from build123d import *

# Parameters (mm, degrees)
BASE_PLATE_DEPTH     = 10
GUIDE_WALL_DEPTH     = 40
HUB_BLOCK_DEPTH      = 40
CLEVIS_START         = -10
CLEVIS_EAR_DEPTH     = 10
GUSSET_SKETCH_W      = 4
GUSSET_SKETCH_H      = 40
GUSSET_DEPTH         = 90
CROSS_HOLE_SKETCH_R  = 8
CROSS_HOLE_16_DEPTH  = 90
HUB_BOSS_SKETCH_R    = 30
HUB_BOSS_60_DEPTH    = 20
HUB_RECESS_SKETCH_R  = 20
HUB_RECESS_40_DEPTH  = 10
SPLINE_BORE_6X_DEPTH = 90


with BuildPart() as part:
    # Base Plate Sketch → Base Plate (new body)
    with BuildSketch(Plane(origin=(0, 0, 0), x_dir=(1, 0, 0), z_dir=(0, 1, 0))):
        with BuildLine():
            Line((-60.5, 45), (60.5, 45))
            ThreePointArc((60.5, 45), (67.571067812, 42.071067812), (70.5, 35))
            Line((70.5, 35), (70.5, -35))
            ThreePointArc((70.5, -35), (67.571067812, -42.071067812), (60.5, -45))
            Line((60.5, -45), (-60.5, -45))
            ThreePointArc((-60.5, -45), (-67.571067812, -42.071067812), (-70.5, -35))
            Line((-70.5, -35), (-70.5, -10))
            Line((-70.5, -10), (-50.5, -10))
            Line((-50.5, -10), (-50.5, 10))
            Line((-50.5, 10), (-70.5, 10))
            Line((-70.5, 10), (-70.5, 35))
            ThreePointArc((-70.5, 35), (-67.571067812, 42.071067812), (-60.5, 45))
        make_face()
    extrude(amount=BASE_PLATE_DEPTH)

    # Guide Wall Sketch → Guide Wall (add)
    with BuildSketch(Plane(origin=(0, 10, 0), x_dir=(1, 0, 0), z_dir=(0, 1, 0))):
        with BuildLine():
            Line((-29.5, 45), (-60.5, 45))
            ThreePointArc((-60.5, 45), (-67.571067812, 42.071067812), (-70.5, 35))
            Line((-70.5, 35), (-70.5, 10))
            Line((-70.5, 10), (-60.5, 10))
            Line((-60.5, 10), (-60.5, 35))
            Line((-60.5, 35), (-29.5, 35))
            Line((-29.5, 35), (-29.5, 45))
        make_face()
        with BuildLine():
            Line((-70.5, -10), (-70.5, -35))
            ThreePointArc((-70.5, -35), (-67.571067812, -42.071067812), (-60.5, -45))
            Line((-60.5, -45), (-29.5, -45))
            Line((-29.5, -45), (-29.5, -35))
            Line((-29.5, -35), (-60.5, -35))
            Line((-60.5, -35), (-60.5, -10))
            Line((-60.5, -10), (-70.5, -10))
        make_face()
    extrude(amount=GUIDE_WALL_DEPTH)

    # Hub Block Sketch → Hub Block (add)
    with BuildSketch(Plane(origin=(0, 10, 0), x_dir=(1, 0, 0), z_dir=(0, 1, 0))):
        with BuildLine():
            Line((45.5, -45), (45.5, 45))
            Line((45.5, 45), (-8.634596738, 28.730536702))
            ThreePointArc((-8.634596738, 28.730536702), (-30, 0), (-8.634596738, -28.730536702))
            Line((-8.634596738, -28.730536702), (45.5, -45))
        make_face()
    extrude(amount=HUB_BLOCK_DEPTH)

    # Clevis Ear Sketch → Clevis Ear (add)
    with BuildSketch(Plane(origin=(0, 50, 0), x_dir=(1, 0, 0), z_dir=(0, 1, 0)).offset(CLEVIS_START)):
        with BuildLine():
            Line((45.5, 45), (60.5, 45))
            ThreePointArc((60.5, 45), (67.571067812, 42.071067812), (70.5, 35))
            Line((70.5, 35), (70.5, -35))
            ThreePointArc((70.5, -35), (67.571067812, -42.071067812), (60.5, -45))
            Line((60.5, -45), (45.5, -45))
            Line((45.5, -45), (45.5, 45))
        make_face()
    extrude(amount=CLEVIS_EAR_DEPTH)

    # Gusset Sketch → Gusset (add)
    with BuildSketch(Plane.XY.offset(45)):
        with Locations((47.5, 30)):
            Rectangle(GUSSET_SKETCH_W, GUSSET_SKETCH_H)
    extrude(amount=-GUSSET_DEPTH)

    # Cross Hole Sketch → Cross Hole Ø16 (cut)
    with BuildSketch(Plane(origin=(0, 50, 0), x_dir=(1, 0, 0), z_dir=(0, 1, 0))):
        with Locations(Location((52.5, 0, 0), (0, 0, 270))):
            Circle(CROSS_HOLE_SKETCH_R)
    extrude(amount=-CROSS_HOLE_16_DEPTH, mode=Mode.SUBTRACT)

    # Hub Boss Sketch → Hub Boss Ø60 (add)
    with BuildSketch(Plane(origin=(0, 50, 0), x_dir=(1, 0, 0), z_dir=(0, 1, 0))):
        with Locations(Location((0, 0, 0), (0, 0, 106.727481019))):
            Circle(HUB_BOSS_SKETCH_R)
    extrude(amount=HUB_BOSS_60_DEPTH)

    # Hub Recess Sketch → Hub Recess Ø40 (cut)
    with BuildSketch(Plane(origin=(0, 70, 0), x_dir=(1, 0, 0), z_dir=(0, 1, 0))):
        with Locations(Location((0, 0, 0), (0, 0, 270))):
            Circle(HUB_RECESS_SKETCH_R)
    extrude(amount=-HUB_RECESS_40_DEPTH, mode=Mode.SUBTRACT)

    # Spline Bore Sketch → Spline Bore 6x (cut)
    with BuildSketch(Plane(origin=(0, 60, 0), x_dir=(1, 0, 0), z_dir=(0, 1, 0))):
        with BuildLine():
            Line((-3.703283788, -11.414275675), (-2.676165673, -9.635254916))
            ThreePointArc((-2.676165673, -9.635254916), (0, -10), (2.676165673, -9.635254916))
            Line((2.676165673, -9.635254916), (3.703283788, -11.414275675))
            Line((3.703283788, -11.414275675), (4.834936491, -13.374355653))
            Line((4.834936491, -13.374355653), (9.165063509, -10.874355653))
            Line((9.165063509, -10.874355653), (8.033410807, -8.914275675))
            Line((8.033410807, -8.914275675), (7.006292692, -7.135254916))
            ThreePointArc((7.006292692, -7.135254916), (8.660254038, -5), (9.682458366, -2.5))
            Line((9.682458366, -2.5), (11.736694594, -2.5))
            Line((11.736694594, -2.5), (14, -2.5))
            Line((14, -2.5), (14, 2.5))
            Line((14, 2.5), (11.736694594, 2.5))
            Line((11.736694594, 2.5), (9.682458366, 2.5))
            ThreePointArc((9.682458366, 2.5), (8.660254038, 5), (7.006292692, 7.135254916))
            Line((7.006292692, 7.135254916), (8.033410807, 8.914275675))
            Line((8.033410807, 8.914275675), (9.165063509, 10.874355653))
            Line((9.165063509, 10.874355653), (4.834936491, 13.374355653))
            Line((4.834936491, 13.374355653), (3.703283788, 11.414275675))
            Line((3.703283788, 11.414275675), (2.676165673, 9.635254916))
            ThreePointArc((2.676165673, 9.635254916), (0, 10), (-2.676165673, 9.635254916))
            Line((-2.676165673, 9.635254916), (-3.703283788, 11.414275675))
            Line((-3.703283788, 11.414275675), (-4.834936491, 13.374355653))
            Line((-4.834936491, 13.374355653), (-9.165063509, 10.874355653))
            Line((-9.165063509, 10.874355653), (-8.033410807, 8.914275675))
            Line((-8.033410807, 8.914275675), (-7.006292692, 7.135254916))
            ThreePointArc((-7.006292692, 7.135254916), (-8.660254038, 5), (-9.682458366, 2.5))
            Line((-9.682458366, 2.5), (-11.736694594, 2.5))
            Line((-11.736694594, 2.5), (-14, 2.5))
            Line((-14, 2.5), (-14, -2.5))
            Line((-14, -2.5), (-11.736694594, -2.5))
            Line((-11.736694594, -2.5), (-9.682458366, -2.5))
            ThreePointArc((-9.682458366, -2.5), (-8.660254038, -5), (-7.006292692, -7.135254916))
            Line((-7.006292692, -7.135254916), (-8.033410807, -8.914275675))
            Line((-8.033410807, -8.914275675), (-9.165063509, -10.874355653))
            Line((-9.165063509, -10.874355653), (-4.834936491, -13.374355653))
            Line((-4.834936491, -13.374355653), (-3.703283788, -11.414275675))
        make_face()
    extrude(amount=-SPLINE_BORE_6X_DEPTH, mode=Mode.SUBTRACT)


solid = part.part
Could you check a few things on this model? Use its own coordinates, in mm. A direction names the side the tool comes from. Give positions to 0.01 mm unless a question says otherwise; leave off trailing zeros. Order: outer loops, then holes, each group sorted by start corner. A loop starts at its lowest first (then second) coordinate and runs counter-clockwise, first axis right, second up. Notation, with made-up numbers: (-24, 71) -> (-13, 71) arc R17 cw to (-13, 84) -> close; hole circle Ø4 at (27.5, 61.25). An arc over 180 degrees is marked (long way). Answer in a Markdown table with one row per item. Add a question column.
Item 1: Imagine slicing it at B-B (z = 0). List the corners of the cut face in (x, y) for me.
Item 2: I'm going to push flat-ended pins straight in: P1, Ø1, axis at x = -3, y = 32.5, coming from the -Z side; P2, Ø1.3, axis at x = -11.5, y = 17.5, coming from the +Z side; P3, Ø8, axis at y = 6, z = 2.5, coming from the -X side. Where does each tip first touch, or does it pass through?
Item 3: Imagine slicing it at D-D (x = -39.5). List the corners of the cut face in (y, z) for me.
Item 4: Imagine slicing it at A-A (x = 52.5). List the corners of the cut face in (y, z) for me.
Item 5: We'd pull the mould along Z, two halves only. Please class faces 4 (the flat face through (18.81, 29.72, -36.98)), 5 (the flat face through (-29.5, 30, 40)), 6 (the flat face through (-30.3, 10, -0.6)): pulls with the +Z half, pulls with the -Z half, needs draft (parallel to the pull), parting line crosses it, or undercut.
Item 6: Please list where these lines run through material, in increasing order: probe 1 along Y at (x, z) = (52, -34); probe 2 along Z at (x, y) = (-54.5, 29.5); probe 3 along X at (y, z) = (9, 12.5).
Item 7: For faces 1 (the flat face through (-70.5, 25, -23)), 2 (the flat face through (-45, 30, 35)), 3 (the cylindrical face through (-8.679, 30.42, 4.967)), which set-ups out of +Z, -Z, +X, -X, +Y, -Y let a thin tool reach every point of the face, with its end or its side?
Item 8: Imagine slicing it at C-C (y = 58). List the corners of the cut face in (x, z) for me.
Result:
| question | item | result |
|---|---|---|
| 1 | outline | (-50.5, 0) -> (-14, 0) -> (-14, 60) -> (-20, 60) -> (-20, 70) -> (-30, 70) -> (-30, 10) -> (-50.5, 10) -> close; (14, 0) -> (44.5, 0) -> (44.5, 50) -> (30, 50) -> (30, 70) -> (20, 70) -> (20, 60) -> (14, 60) -> close; (60.5, 0) -> (70.5, 0) -> (70.5, 10) -> (60.5, 10) -> close; (60.5, 40) -> (70.5, 40) -> (70.5, 50) -> (60.5, 50) -> close |
| 2 | P1 | z = -30.57 |
| 2 | P2 | z = 27.97 |
| 2 | P3 | x = -50.5 |
| 3 | outline | (0, -45) -> (50, -45) -> (50, -35) -> (10, -35) -> (10, 35) -> (50, 35) -> (50, 45) -> (0, 45) -> close |
| 4 | outline | (0, -45) -> (10, -45) -> (10, -8) -> (0, -8) -> close; (0, 8) -> (10, 8) -> (10, 45) -> (0, 45) -> close; (40, -45) -> (50, -45) -> (50, -8) -> (40, -8) -> close; (40, 8) -> (50, 8) -> (50, 45) -> (40, 45) -> close |
| 5 | face 4 | pulls with the -Z half |
| 5 | face 5 | needs draft |
| 5 | face 6 | undercut |
| 6 | probe 1 | 0 to 10, 40 to 50 |
| 6 | probe 2 | -45 to -35, 35 to 45 |
| 6 | probe 3 | -70.5 to -6.35, -4.33 to 4.33, 6.35 to 70.5 |
| 7 | face 1 | +Z, -Z, -X, +Y, -Y |
| 7 | face 2 | +Y |
| 7 | face 3 | +Y, -Y |
| 8 | outline | circle Ø60 at (0, 0); hole (-14, -2.5) -> (-9.68, -2.5) arc R10 ccw to (-7.01, -7.14) -> (-9.17, -10.87) -> (-4.83, -13.37) -> (-2.68, -9.64) arc R10 ccw to (2.68, -9.64) -> (4.83, -13.37) -> (9.17, -10.87) -> (7.01, -7.14) arc R10 ccw to (9.68, -2.5) -> (14, -2.5) -> (14, 2.5) -> (9.68, 2.5) arc R10 ccw to (7.01, 7.14) -> (9.17, 10.87) -> (4.83, 13.37) -> (2.68, 9.64) arc R10 ccw to (-2.68, 9.64) -> (-4.83, 13.37) -> (-9.17, 10.87) -> (-7.01, 7.14) arc R10 ccw to (-9.68, 2.5) -> (-14, 2.5) -> close |
